```python
from build123d import *

# Parameters (mm, degrees)
SKETCH_1_W                = 23
SKETCH_1_H                = 22
EXTRUDE_1_DEPTH           = 340
HOLE_WIZARD_1_D           = 6.6
HOLE_WIZARD_1_CBORE_D     = 11
HOLE_WIZARD_1_CBORE_DEPTH = 6.8
PATTERN_LINEAR_2_COUNT    = 6
PATTERN_LINEAR_2_PITCH    = 60


with BuildPart() as part:
    # 草图1 → 凸台-拉伸1 (new body)
    with BuildSketch(Plane(origin=(0, 0, 0), x_dir=(0, 0, -1), z_dir=(1, 0, 0))):
        Rectangle(SKETCH_1_W, SKETCH_1_H)
    extrude(amount=EXTRUDE_1_DEPTH)

    # 打孔尺寸(%根据)内六角圆柱头螺钉的类型1 (through all)
    with Locations(Plane(origin=(0, 11, 0), x_dir=(1, 0, 0), z_dir=(0, 1, 0))):
        with Locations((20, 0)):
            hole_wizard_1 = CounterBoreHole(HOLE_WIZARD_1_D / 2, HOLE_WIZARD_1_CBORE_D / 2, HOLE_WIZARD_1_CBORE_DEPTH)

    # 阵列(线性)2: 打孔尺寸(%根据)内六角圆柱头螺钉的类型1 ×6
    with Locations(*[(i * PATTERN_LINEAR_2_PITCH, 0, 0) for i in range(1, PATTERN_LINEAR_2_COUNT)]):
        add(hole_wizard_1, mode=Mode.SUBTRACT)


solid = part.part
```
Verification items for the finished model (mm, model axes). A direction names the side the tool comes from. Coordinates: 2 decimals unless noted, no trailing zeros. Loops run counter-clockwise (first coordinate to the right, second up) from the corner with the lowest first, then second, coordinate; pieces in that order, holes last. Notation, with made-up numbers: (-28, -7) - (-10, -7) arc R29 ccw to (-10, 30) - close; hole circle Ø1 at (28.5, 25.25). An arc over 180 degrees is marked (long way). Put each result on its own line as item: value.
Item 1: Section check C-C (z = 0). Give the number of separate pieces and of enclosed holes in the cut face, then the cut area to 3 significant figures.
Conclusion:
separate pieces: 7
enclosed holes: 0
area: 6,430 mm2
Item 2: Section check B-B (y = -1). Enter the section's corners in (x, z).
Conclusion:
outline: (0, -11.5) - (340, -11.5) - (340, 11.5) - (0, 11.5) - close; hole circle Ø6.6 at (20, 0); hole circle Ø6.6 at (80, 0); hole circle Ø6.6 at (140, 0); hole circle Ø6.6 at (200, 0); hole circle Ø6.6 at (260, 0); hole circle Ø6.6 at (320, 0)
Item 3: Draft check along Z on faces 3 (the face through (316.85, -3.51, -0.99)), 4 (the face through (168, 0, -11.5)), 5 (the face through (168, 11, 0)). Enter one of: pulls with the +Z half, pulls with the -Z half, needs draft (parallel to the pull), parting line crosses it, or undercut.
Conclusion:
face 3: undercut
face 4: pulls with the -Z half
face 5: needs draft
Item 4: Scan lines: line 1 along Z through (x, y) = (320, 9.75); line 2 along Z through (x, y) = (80, -5); line 3 along Y through (x, z) = (22, -3.5). Record each from-to range of solid material in increasing order.
Conclusion:
line 1: z = -11.5 to -5.5, 5.5 to 11.5
line 2: z = -11.5 to -3.3, 3.3 to 11.5
line 3: y = -11 to 4.2
Item 5: Gauge pin test, flat ends, axial feed: pin 1 Ø6 at (x, z) = (80, 0) entering from -Y; pin 2 Ø3.5 at (x, z) = (82.5, 0) entering from +Y. Record the tip position at first contact, or that the pin passes through.
Conclusion:
pin 1: passes through
pin 2: stops at y = 4.2
Item 6: Set-up check for faces 1 (the face through (264, 4.2, 0)), 2 (the face through (16.95, -3.51, 1.26)): record each of +Z, -Z, +X, -X, +Y, -Y from which the full face is reachable in a straight line by a thin tool's end or side.
Conclusion:
face 1: +Y
face 2: +Y, -Y
Item 7: Section check A-A (x = 320). Enter the section's corners in (y, z), then the cut area to 3 significant figures.
Conclusion:
outline: (-11, -11.5) - (11, -11.5) - (11, -5.5) - (4.2, -5.5) - (4.2, -3.3) - (-11, -3.3) - close; (-11, 3.3) - (4.2, 3.3) - (4.2, 5.5) - (11, 5.5) - (11, 11.5) - (-11, 11.5) - close
area: 331 mm2
